Drawing for the job (mm, zero at the part's lowest x, y, z). Give positions to 0.01 mm unless a question says otherwise; leave off trailing zeros. Loops run counter-clockwise (first coordinate to the right, second up) from the corner with the lowest first, then second, coordinate; pieces in that order, holes last. Notation, with made-up numbers: (85, 80.5) - (131, 80.5) arc R22 cw to (131, 118.5) - close; hole circle Ø4 at (31.25, 52.25). An arc over 180 degrees is marked (long way). Return JSON: item names as keys, results as strings. Group by question number.
1) Mould opens along Z. For the marked faces 1, 2 and 3 say: released by +Z, released by -Z, zero draft, split by the parting line, or undercut.
2) Drop flat-ended pins along their axis: pin 1 (0.8 mm diameter, centred on x = 38, y = 0.5, fed in from -Z); pin 2 (4 mm diameter, centred on x = 21.5, y = 4, fed in from +Z); pin 3 (0.5 mm diameter, centred on x = 38.5, y = 0.5, fed in from +Z). Give the stop position or say it passes through.
3) Slice it at C-C (x = 34.5). List the corners of the cut face in (y, z) (1 decimal).
4) Drill centre lines: probe 1 along X at (y, z) = (2, 21.5); probe 2 along Y at (x, z) = (4, 19.5); probe 3 along Z at (x, y) = (27, 4.75). Where is each one in solid material? Low to high. Write a range as from..to.
5) Slice it at B-B (x = 21.5). List the corners of the cut face in (y, z).
6) Slice it at A-A (z = 21.5). List the corners of the cut face in (x, y).
7) Slice it at D-D (y = 4). List the corners of the cut face in (x, z), and give its area (3 significant figures).
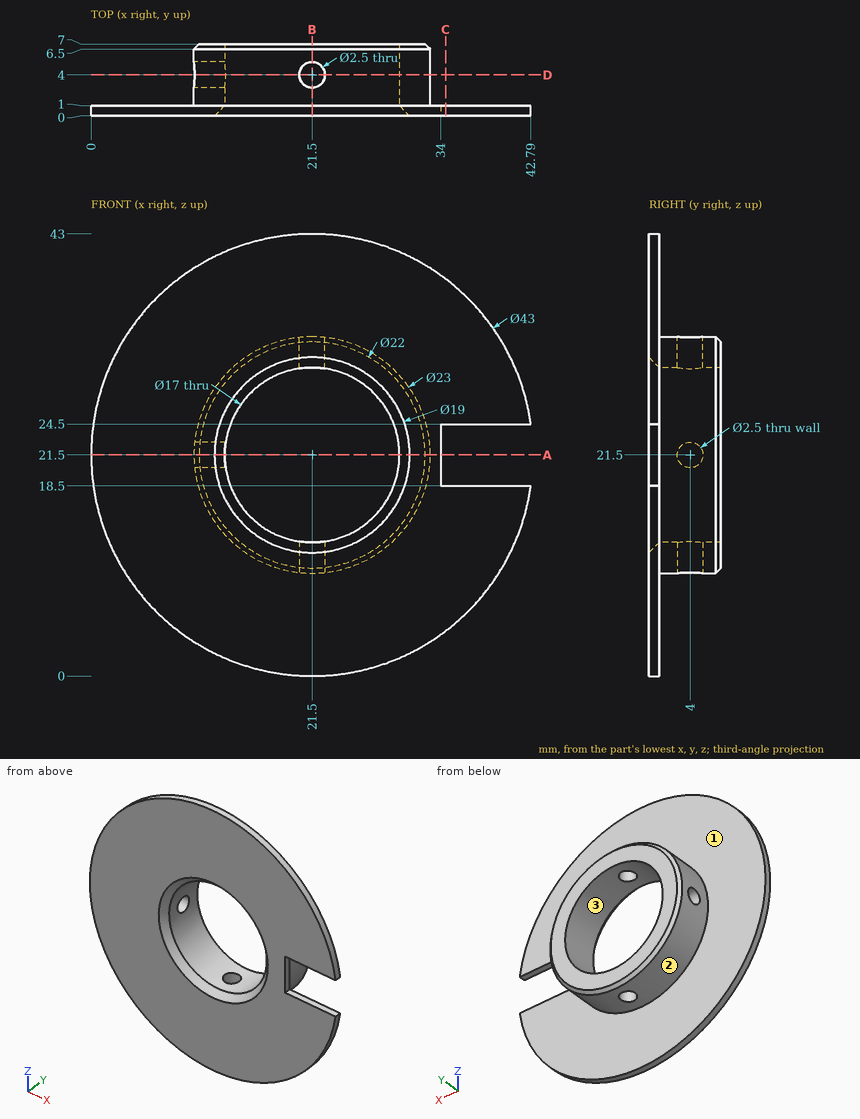
Results:
{
 "1": {"face 1": "zero draft", "face 2": "split by the parting line", "face 3": "undercut"},
 "2": {"pin 1": "z = 7.25", "pin 2": "z = 33", "pin 3": "z = 34.98"},
 "3": {"outline": "(0, 4.4) - (1, 4.4) - (1, 18.5) - (0, 18.5) - close; (0, 24.5) - (1, 24.5) - (1, 38.6) - (0, 38.6) - close"},
 "4": {"probe 1": "10..13, 30..33", "probe 2": "0..1", "probe 3": "11.4..15.02, 27.98..31.6"},
 "5": {"outline": "(0, 0) - (1, 0) - (1, 10) - (2.75, 10) - (2.75, 13) - (1, 13) - (0, 12) - close; (0, 31) - (1, 30) - (2.75, 30) - (2.75, 33) - (1, 33) - (1, 43) - (0, 43) - close; (5.25, 10) - (6.5, 10) - (7, 10.5) - (7, 13) - (5.25, 13) - close; (5.25, 30) - (7, 30) - (7, 32.5) - (6.5, 33) - (5.25, 33) - close"},
 "6": {"outline": "(0, 0) - (12, 0) - (13, 1) - (13, 2.75) - (10, 2.75) - (10, 1) - (0, 1) - close; (10, 5.25) - (13, 5.25) - (13, 7) - (10.5, 7) - (10, 6.5) - close; (30, 1) - (31, 0) - (34, 0) - (34, 1) - (33, 1) - (33, 6.5) - (32.5, 7) - (30, 7) - close"},
 "7": {"outline": "(10.07, 20.25) arc R11.5 ccw to (20.25, 10.07) - (20.25, 13.09) arc R8.5 cw to (13.09, 20.25) - close; (10.07, 22.75) - (13.09, 22.75) arc R8.5 cw to (20.25, 29.91) - (20.25, 32.93) arc R11.5 ccw to start; (22.75, 10.07) arc R11.5 ccw to (22.75, 32.93) - (22.75, 29.91) arc R8.5 cw to (22.75, 13.09) - close", "area": "166 mm2"}
}
